Job drawing, mm, ordinate dimensions from the low corner. One solid piece. Give positions to 0.01 mm unless a question says otherwise; leave off trailing zeros. Order: outer loops, then holes, each group sorted by start corner. A loop starts at its lowest first (then second) coordinate and runs counter-clockwise, first axis right, second up.
1. Slice it at D-D on y = 4.5. List the corners of the cut face in (x, z).
2. Slice it at B-B on y = 8. List the corners of the cut face in (x, z), and give its area (3 significant figures).
3. Probe line 1 (Z direction, x = 4, y = 2.5); line 2 (Y direction, x = 12, z = 2); line 3 (X direction, y = 5, z = 5.25). List the from-to ranges inside material, lowest first.
4. Drop a flat-ended pin along its axis: pin 1 Ø3.5 at (x, z) = (4, 4) entering from +Y. Give the stop position or say it passes through.
5. Slice it at C-C on x = 4. List the corners of the cut face in (y, z), and give its area (3 significant figures).
6. Slice it at A-A on z = 4. List the corners of the cut face in (x, y).
7. Mould opens along Z. For the marked faces 1, 2 and 3 say: +Z half, -Z half, draft (parallel to the pull), parting line (faces both ways), or undercut.
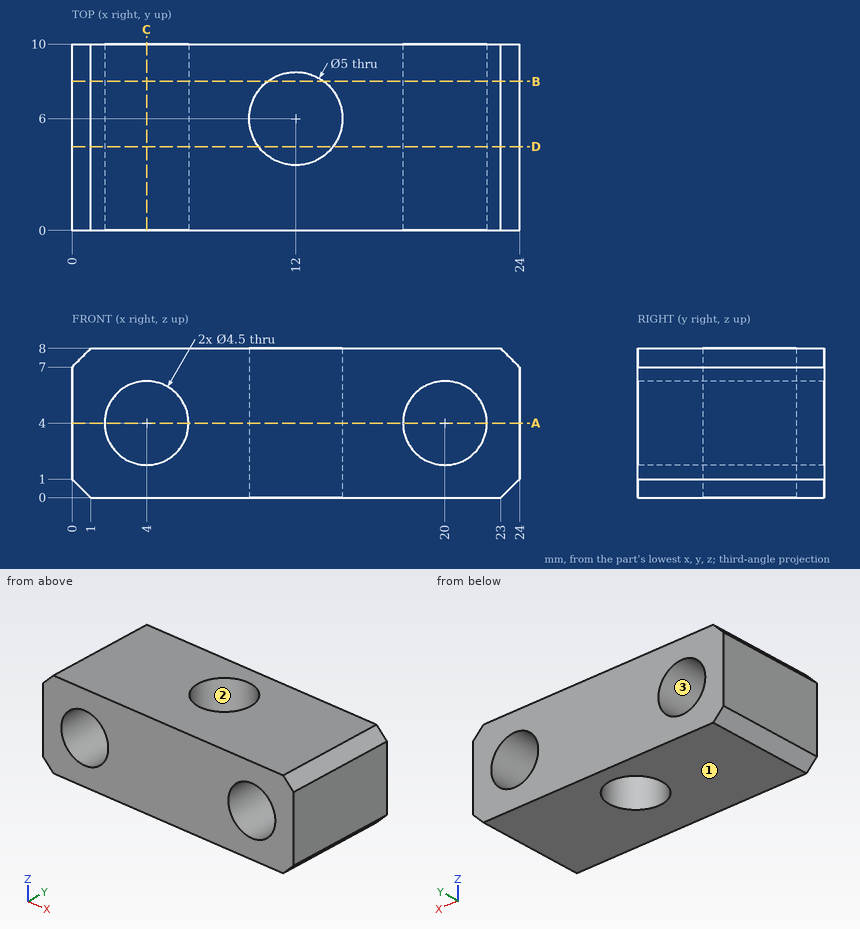
Data:
1. outline: (0, 1) - (1, 0) - (10, 0) - (10, 8) - (1, 8) - (0, 7) - close; (14, 0) - (23, 0) - (24, 1) - (24, 7) - (23, 8) - (14, 8) - close; hole circle Ø4.5 at (4, 4); hole circle Ø4.5 at (20, 4)
2. outline: (0, 1) - (1, 0) - (10.5, 0) - (10.5, 8) - (1, 8) - (0, 7) - close; (13.5, 0) - (23, 0) - (24, 1) - (24, 7) - (23, 8) - (13.5, 8) - close; hole circle Ø4.5 at (4, 4); hole circle Ø4.5 at (20, 4)
2. area: 134 mm2
3. line 1: z = 0 to 1.75, 6.25 to 8
3. line 2: y = 0 to 3.5, 8.5 to 10
3. line 3: x = 0 to 2.13, 5.87 to 9.71, 14.29 to 18.13, 21.87 to 24
4. pin 1: passes through
5. outline: (0, 0) - (10, 0) - (10, 1.75) - (0, 1.75) - close; (0, 6.25) - (10, 6.25) - (10, 8) - (0, 8) - close
5. area: 35.0 mm2
6. outline: (0, 0) - (1.75, 0) - (1.75, 10) - (0, 10) - close; (6.25, 0) - (17.75, 0) - (17.75, 10) - (6.25, 10) - close; (22.25, 0) - (24, 0) - (24, 10) - (22.25, 10) - close; hole circle Ø5 at (12, 6)
7. face 1: -Z half
7. face 2: draft
7. face 3: undercut
